```python
from build123d import *

# Parameters (mm, degrees)
SKETCH1_R           = 10
BOSS_EXTRUDE1_DEPTH = 15


with BuildPart() as part:
    # Sketch1 → Boss-Extrude1 (new body)
    with BuildSketch(Plane(origin=(0, 0, 0), x_dir=(1, 0, 0), z_dir=(0, 1, 0))):
        with BuildLine():
            Line((-20, 0), (-20, 250))
            ThreePointArc((-20, 250), (0, 270), (20, 250))
            Line((20, 250), (20, 0))
            ThreePointArc((20, 0), (0, -20), (-20, 0))
        make_face()
        with Locations(Location((0, 250, 0), (0, 0, 270))):
            Circle(SKETCH1_R, mode=Mode.SUBTRACT)
        with Locations(Location((0, 0, 0), (0, 0, 270))):
            Circle(SKETCH1_R, mode=Mode.SUBTRACT)
    extrude(amount=BOSS_EXTRUDE1_DEPTH)


solid = part.part
```
Model file for the job. Use its own axes, mm. Coordinates: 2 decimals unless noted, no trailing zeros. Loops run counter-clockwise (first coordinate to the right, second up) from the corner with the lowest first, then second, coordinate; pieces in that order, holes last. Notation, with made-up numbers: (-19, 80.5) -> (1, 80.5) arc R19 ccw to (1, 111.5) -> close; hole circle Ø10 at (-32.5, 11). An arc over 180 degrees is marked (long way). Answer as a JSON object with one key per item and string values.
Q1. Flat gauge pins, fed straight in: P1, Ø1.5, axis at x = 7, y = 4.5, coming from the +Z side; P2, Ø2, axis at x = -11, y = 11.5, coming from the +Z side; P3, Ø4, axis at x = 2.5, y = 3, coming from the +Z side. Where does each tip first touch, or does it go through?
Report:
{"P1": "stops at z = 19", "P2": "stops at z = 17.32", "P3": "stops at z = 19.99"}
Q2. Probe probe 1 along Z at (x, y) = (2, 11); probe 2 along Z at (x, y) = (-8, 2.75); probe 3 along X at (y, z) = (5, -250). List the from-to ranges inside material, lowest first.
Report:
{"probe 1": "z = -269.9 to -259.8, -240.2 to -9.8, 9.8 to 19.9", "probe 2": "z = -268.33 to -256, -244 to -6, 6 to 18.33", "probe 3": "x = -20 to -10, 10 to 20"}
Q3. Cut at D-D (x = 16). List the corners of the cut face in (y, z), and give its area (3 significant figures).
Report:
{"outline": "(0, -262) -> (15, -262) -> (15, 12) -> (0, 12) -> close", "area": "4,110 mm2"}
Q4. Cut at A-A (x = 0). List the corners of the cut face in (y, z), and give its area (3 significant figures).
Report:
{"outline": "(0, -270) -> (15, -270) -> (15, -260) -> (0, -260) -> close; (0, -240) -> (15, -240) -> (15, -10) -> (0, -10) -> close; (0, 10) -> (15, 10) -> (15, 20) -> (0, 20) -> close", "area": "3,750 mm2"}
Q5. Cut at C-C (y = 8.75). List the corners of the cut face in (x, z).
Report:
{"outline": "(-20, -250) arc R20 ccw to (20, -250) -> (20, 0) arc R20 ccw to (-20, 0) -> close; hole circle Ø20 at (0, -250); hole circle Ø20 at (0, 0)"}
Q6. Cut at B-B (z = -246.5). List the corners of the cut face in (x, y).
Report:
{"outline": "(-20, 0) -> (-9.37, 0) -> (-9.37, 15) -> (-20, 15) -> close; (9.37, 0) -> (20, 0) -> (20, 15) -> (9.37, 15) -> close"}
Q7. Pull direction X, two halves, no side cores. Call faces 1 (the flat face through (-20, 7, -123)), 2 (the cylindrical face through (0, 7, -270)), 3 (the cylindrical face through (-3.83, 7.395, -240.763)): released by +X, released by -X, zero draft, split by the parting line, or undercut.
Report:
{"face 1": "released by -X", "face 2": "split by the parting line", "face 3": "undercut"}
